Could you check a few things on this drawing? It's one solid part, dimensions in mm from its lowest x, y, z. A direction names the side the tool comes from. Round coordinates to 2 decimals unless told otherwise and drop trailing zeros. Write each loop counter-clockwise with the first axis right and the second up, starting at its lowest first coordinate (ties: lowest second). Pieces come first, ordered by that corner, then holes. Notation, with made-up numbers: (21, 41.5) - (80, 41.5) arc R30 ccw to (80, 75.5) - close; hole circle Ø10 at (15, -1). An arc over 180 degrees is marked (long way). Use one line per item in the form item = value. Start each with the question number.
1. I want a section at B-B, the plane z = 12.25. List the corners of the cut face in (x, y) for me, plus the area to 3 significant figures.
2. Which directions (+Z, -Z, +X, -X, +Y, -Y) give clear straight access to the entire face, cutting with the end or side of a thin tool? Please do the marked faces 4 and 5.
3. If I drill on line 1 along X through (y, z) = (56.5, 21.25); line 2 along Y through (x, z) = (184.5, 17.25), over which ranges is the centre line in solid material (lowest first)?
4. I want a section at C-C, the plane x = 182. List the corners of the cut face in (y, z) for me, plus the area to 3 significant figures.
5. Will this pin go through, and if not, where does the flat tip stop? pin 1 (12.5 mm diameter, centred on x = 155, z = 11, fed in from -Y).
6. I want a section at A-A, the plane y = 19. List the corners of the cut face in (x, z) for me.
7. We'd pull the mould along X, two halves only. Please class the marked faces 1, 2 and 3: +X half, -X half, draft (parallel to the pull), parting line (faces both ways), or undercut.
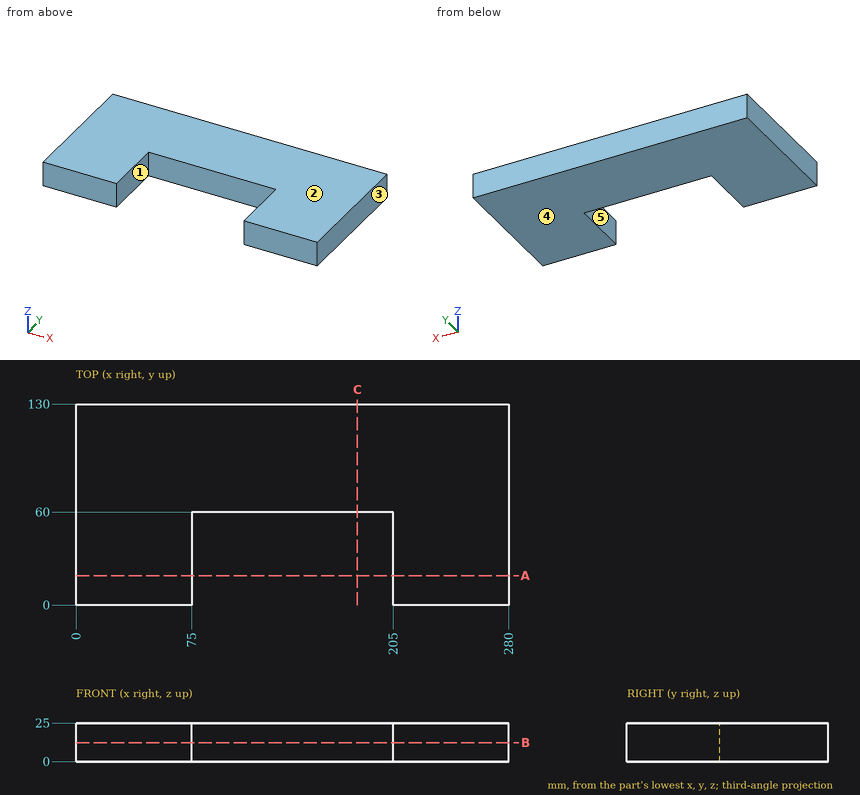
Model answer:
q1.outline = (0, 0) - (75, 0) - (75, 60) - (205, 60) - (205, 0) - (280, 0) - (280, 130) - (0, 130) - close
q1.area = 28,600 mm2
q2.face_4 = -Z, +X, -X, +Y, -Y
q2.face_5 = +Z, -Z, -Y
q3.line_1 = 0 to 75, 205 to 280
q3.line_2 = 60 to 130
q4.outline = (60, 0) - (130, 0) - (130, 25) - (60, 25) - close
q4.area = 1,750 mm2
q5.pin_1 = 60
q6.outline = (0, 0) - (75, 0) - (75, 25) - (0, 25) - close; (205, 0) - (280, 0) - (280, 25) - (205, 25) - close
q7.face_1 = undercut
q7.face_2 = draft
q7.face_3 = +X half
